The drawing under review shows one solid part. Ordinate dimensions are in mm from its lowest x, y, z. A direction names the side the tool comes from. Round coordinates to 2 decimals unless told otherwise and drop trailing zeros. Order: outer loops, then holes, each group sorted by start corner. A loop starts at its lowest first (then second) coordinate and runs counter-clockwise, first axis right, second up.
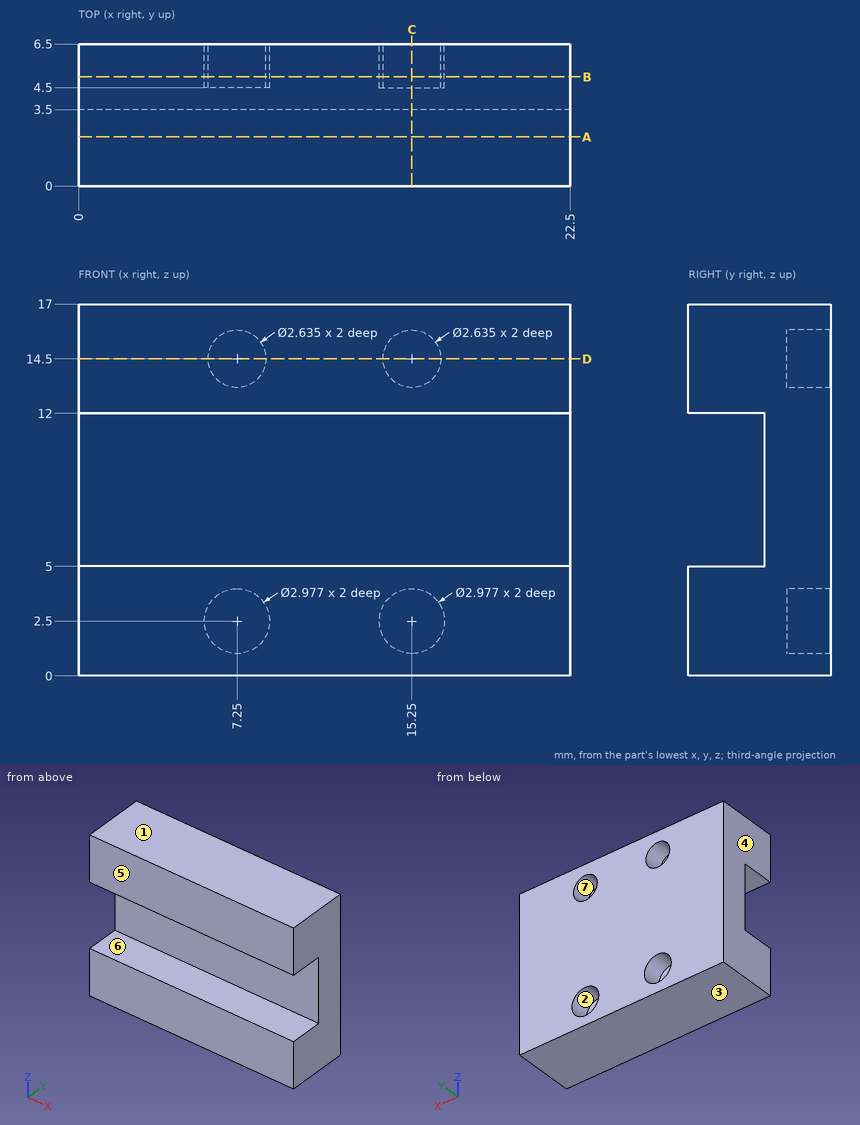
(1) We need section A-A (y = 2.25). Give the boundary of the cut face in (x, z).
(2) To check wall thickness, follow L1, parallel to X at y = 5.4, z = 2.5; L2, parallel to Z at x = 8.5, y = 2; L3, parallel to X at y = 5.8, z = 14.5. State the ranges of each line that lie inside material, in increasing order.
(3) Tool access review of the marked faces 5, 6 and 7: name each direction out of +Z, -Z, +X, -X, +Y, -Y from which nothing blocks a thin tool from reaching the whole face with its end or side.
(4) Clearance check with flat-ended pins moving along their axes: P1, Ø5.5, axis at x = 6, z = 9, coming from the -Y side; P2, Ø0.9, axis at x = 7.5, z = 2, coming from the +Y side. State where each tip first meets the part, or that it passes through.
(5) We need section D-D (z = 14.5). Give the boundary of the cut face in (x, y), and give its area (3 significant figures).
(6) The part is to be moulded in two halves that separate along Z. For the marked faces 1, 2, 3 and 4, say which applies: pulls with the +Z half, pulls with the -Z half, needs draft (parallel to the pull), parting line crosses it, or undercut.
(7) We need section C-C (x = 15.25). Give the boundary of the cut face in (y, z), and give its area (3 significant figures).
(8) We need section B-B (y = 5). Count the separate pieces of the cut face and the enclosed holes in it, and give its area (3 significant figures).
Verdict:
1. outline: (0, 0) - (22.5, 0) - (22.5, 5) - (0, 5) - close; (0, 12) - (22.5, 12) - (22.5, 17) - (0, 17) - close
2. L1: x = 0 to 5.76, 8.74 to 13.76, 16.74 to 22.5
2. L2: z = 0 to 5, 12 to 17
2. L3: x = 0 to 5.93, 8.57 to 13.93, 16.57 to 22.5
3. face 5: +Z, -Z, +X, -X, -Y
3. face 6: +X, -X, -Y
3. face 7: +Y
4. P1: stops at y = 3.5
4. P2: stops at y = 4.5
5. outline: (0, 0) - (22.5, 0) - (22.5, 6.5) - (16.57, 6.5) - (16.57, 4.5) - (13.93, 4.5) - (13.93, 6.5) - (8.57, 6.5) - (8.57, 4.5) - (5.93, 4.5) - (5.93, 6.5) - (0, 6.5) - close
5. area: 136 mm2
6. face 1: pulls with the +Z half
6. face 2: undercut
6. face 3: pulls with the -Z half
6. face 4: needs draft
7. outline: (0, 0) - (6.5, 0) - (6.5, 1.01) - (4.5, 1.01) - (4.5, 3.99) - (6.5, 3.99) - (6.5, 13.18) - (4.5, 13.18) - (4.5, 15.82) - (6.5, 15.82) - (6.5, 17) - (0, 17) - (0, 12) - (3.5, 12) - (3.5, 5) - (0, 5) - close
7. area: 74.8 mm2
8. separate pieces: 1
8. enclosed holes: 4
8. area: 358 mm2
